from build123d import *

# Parameters (mm, degrees)
EXTRUDE_THIN1_DEPTH = 484.14
FILLET1_R           = 5
FILLET2_R           = 1.333333333
SKETCH2_W           = 36
SKETCH2_H           = 41
CUT_EXTRUDE1_DEPTH  = 488.43362584
SKETCH3_W           = 36
SKETCH3_H           = 41
CUT_EXTRUDE3_DEPTH  = 488.43362584
CUT_EXTRUDE4_DEPTH  = 14
LPATTERN1_COUNT     = 2
LPATTERN1_PITCH     = 287.14


with BuildPart() as part:
    # Sketch1 → Extrude-Thin1 (new body)
    with BuildSketch(Plane.XY):
        Polygon((0, 40), (0, 0), (40, 0), (40, 4), (4, 4), (4, 40), align=None)
    extrude(amount=EXTRUDE_THIN1_DEPTH)

    # Fillet1
    fillet1_edges = [part.edges().sort_by_distance(p)[0] for p in [
        (4, 4, 242.07),
    ]]
    fillet(fillet1_edges, radius=FILLET1_R)

    # Fillet2
    fillet2_edges = [part.edges().sort_by_distance(p)[0] for p in [
        (40, 4, 242.07),
        (4, 40, 242.07),
    ]]
    fillet(fillet2_edges, radius=FILLET2_R)

    # Sketch2 → Cut-Extrude1 (cut, through all)
    with BuildSketch(Plane.XZ):
        with Locations((22, 20.5)):
            Rectangle(SKETCH2_W, SKETCH2_H)
    extrude(amount=-CUT_EXTRUDE1_DEPTH, mode=Mode.SUBTRACT)

    # Sketch3 → Cut-Extrude3 (cut, through all)
    with BuildSketch(Plane.XZ):
        with Locations((22, 463.64)):
            Rectangle(SKETCH3_W, SKETCH3_H)
    extrude(amount=-CUT_EXTRUDE3_DEPTH, mode=Mode.SUBTRACT)

    # Sketch4 → Cut-Extrude4 (cut)
    with BuildSketch(Plane(origin=(4, 0, 0), x_dir=(0, 0, -1), z_dir=(1, 0, 0))):
        with BuildLine():
            Line((-391.14, 32), (-377.14, 32))
            ThreePointArc((-377.14, 32), (-370.14, 25), (-377.14, 18))
            Line((-377.14, 18), (-391.14, 18))
            ThreePointArc((-391.14, 18), (-398.14, 25), (-391.14, 32))
        make_face()
    cut_extrude4 = extrude(amount=-CUT_EXTRUDE4_DEPTH, mode=Mode.SUBTRACT)

    # LPattern1: Cut-Extrude4 ×2
    with Locations(*[(0, 0, -i * LPATTERN1_PITCH) for i in range(1, LPATTERN1_COUNT)]):
        add(cut_extrude4, mode=Mode.SUBTRACT)


solid = part.part
For this review, take the finished solid that the model builds, in its own axes (mm). A direction names the side the tool comes from. Give positions to 0.01 mm unless a question says otherwise; leave off trailing zeros. Order: outer loops, then holes, each group sorted by start corner. A loop starts at its lowest first (then second) coordinate and runs counter-clockwise, first axis right, second up. Notation, with made-up numbers: (-20.5, 19) - (35.5, 19) arc R13 ccw to (35.5, 42) - close; hole circle Ø9 at (16, 77.5). An arc over 180 degrees is marked (long way). Answer as a JSON object with one key per item and string values. Group by question number.
Item 1: Machinability: for faces 1 (the flat face through (22, 2, 443.14)), 2 (the flat face through (0, 20, 239)), 3 (the flat face through (20, 0, 239)), 4 (the flat face through (24, 4, 239)), 5 (the flat face through (22, 2, 41)), which of the approach directions +Z, -Z, +X, -X, +Y, -Y give a long, thin tool a straight path to every point of the face, cutting with its end or side? Answer none if there is none.
Item 2: Clearance check with flat-ended pins moving along their axes: pin 1 Ø23.5 at (x, z) = (21.5, 177.5) entering from +Y; pin 2 Ø8 at (y, z) = (7.5, 91) entering from +X; pin 3 Ø5 at (y, z) = (12.5, 398.5) entering from +X; pin 4 Ø4.5 at (x, y) = (15, 6.5) entering from +Z. State where each tip first meets the part, or that it passes through.
Item 3: Take a section at B-B on y = 27.5. Give the boundary of the cut face in (x, z), and give its area (3 significant figures).
Item 4: Take a section at C-C on z = 190. Give the boundary of the cut face in (x, y), and give its area (3 significant figures).
Item 5: Take a section at A-A on z = 94.5. Give the boundary of the cut face in (x, y), and give its area (3 significant figures).
Item 6: Take a section at D-D on x = 14. Give the boundary of the cut face in (y, z).
Item 7: Wall thickness on line 1 along Y through (x, z) = (10.5, 384.5); line 2 along Z through (x, y) = (27, 3.5): over which ranges is each line inside the solid? List them lowest first.
Reported:
{
 "1": {"face 1": "+Z, +X, +Y, -Y", "face 2": "+Z, -Z, -X, +Y, -Y", "face 3": "+Z, -Z, +X, -X, -Y", "face 4": "+Z, -Z, +X, +Y", "face 5": "-Z, +X, +Y, -Y"},
 "2": {"pin 1": "y = 4", "pin 2": "x = 39.71", "pin 3": "x = 4", "pin 4": "through"},
 "3": {"outline": "(0, 0) - (4, 0) - (4, 83.46) - (0, 83.46) - close; (0, 110.54) - (4, 110.54) - (4, 370.6) - (0, 370.6) - close; (0, 397.68) - (4, 397.68) - (4, 484.14) - (0, 484.14) - close", "area": "1,720 mm^2"},
 "4": {"outline": "(0, 0) - (40, 0) - (40, 2.67) arc R1.33 ccw to (38.67, 4) - (9, 4) arc R5 cw to (4, 9) - (4, 38.67) arc R1.33 ccw to (2.67, 40) - (0, 40) - close", "area": "309 mm^2"},
 "5": {"outline": "(0, 0) - (40, 0) - (40, 2.67) arc R1.33 ccw to (38.67, 4) - (9, 4) arc R5 cw to (4, 9) - (4, 18) - (0, 18) - close; (0, 32) - (4, 32) - (4, 38.67) arc R1.33 ccw to (2.67, 40) - (0, 40) - close", "area": "253 mm^2"},
 "6": {"outline": "(0, 41) - (4, 41) - (4, 443.14) - (0, 443.14) - close"},
 "7": {"line 1": "0 to 4", "line 2": "41 to 443.14"}
}
